Part model, mm, in its own coordinate system. A direction names the side the tool comes from. Round coordinates to 2 decimals unless told otherwise and drop trailing zeros. Write each loop counter-clockwise with the first axis right and the second up, starting at its lowest first coordinate (ties: lowest second). Pieces come first, ordered by that corner, then holes.
from build123d import *

# Parameters (mm, degrees)
BASE_BODY_DEPTH              = 37.5
UPPER_FLANGE_DEPTH           = 75
FLANGE_CORNER_FILLET_R13_A_R = 13
FLANGE_CORNER_FILLET_R13_B_R = 13
MOUNTING_HOLES_SKETCH_R      = 5
MOUNTING_HOLES_2X_10_DEPTH   = 75
SLOT_6MM_DEPTH               = 75
HANGER_PLATE_DEPTH           = 75
TAPER_CUT_DEPTH              = 75
EYE_BOSS_SKETCH_R            = 25
EYE_BOSS_DEPTH               = 10
EYE_HOLE_SKETCH_R            = 11.5
EYE_HOLE_23_DEPTH            = 10


with BuildPart() as part:
    # Base Profile Sketch → Base Body (new, symmetric)
    with BuildSketch(Plane.XY):
        Polygon((0, 11), (0, 21), (-27, 21), (-27, -21), (0, -21), (0, -11), (-17, -11), (-17, 11), align=None)
    extrude(amount=BASE_BODY_DEPTH, both=True)

    # Upper Flange Sketch → Upper Flange (add)
    with BuildSketch(Plane.XY.offset(37.5)):
        Polygon((0, 21), (0, 54), (10, 54), (10, 21), (10, 6.5), (0, 6.5), align=None)
    extrude(amount=-UPPER_FLANGE_DEPTH)

    # Flange Corner Fillet R13 A
    flange_corner_fillet_r13_a_edges = [part.edges().sort_by_distance(p)[0] for p in [
        (5, 54, 37.5),
    ]]
    fillet(flange_corner_fillet_r13_a_edges, radius=FLANGE_CORNER_FILLET_R13_A_R)

    # Flange Corner Fillet R13 B
    flange_corner_fillet_r13_b_edges = [part.edges().sort_by_distance(p)[0] for p in [
        (5, 54, -37.5),
    ]]
    fillet(flange_corner_fillet_r13_b_edges, radius=FLANGE_CORNER_FILLET_R13_B_R)

    # Mounting Holes Sketch → Mounting Holes 2xØ10 (cut)
    with BuildSketch(Plane.ZY):
        with Locations((24.5, 41)):
            Circle(MOUNTING_HOLES_SKETCH_R)
        with Locations((-24.5, 41)):
            Circle(MOUNTING_HOLES_SKETCH_R)
    extrude(amount=-MOUNTING_HOLES_2X_10_DEPTH, mode=Mode.SUBTRACT)

    # Slot Sketch → Slot 6mm (cut)
    with BuildSketch(Plane.ZY.offset(27)):
        with BuildLine():
            Line((-17.5, 6), (17.5, 6))
            ThreePointArc((17.5, 6), (23.5, 0), (17.5, -6))
            Line((17.5, -6), (-17.5, -6))
            ThreePointArc((-17.5, -6), (-23.5, 0), (-17.5, 6))
        make_face()
    extrude(amount=-SLOT_6MM_DEPTH, mode=Mode.SUBTRACT)

    # Hanger Plate Sketch → Hanger Plate (add)
    with BuildSketch(Plane.XY.offset(37.5)):
        Polygon((0, -6.5), (0, -21), (0, -73), (10, -73), (10, -21), (10, -6.5), align=None)
    extrude(amount=-HANGER_PLATE_DEPTH)

    # Taper Cut Sketch → Taper Cut (cut)
    with BuildSketch(Plane.ZY):
        Polygon((37.5, -73), (37.5, -21), (25, -73), align=None)
        Polygon((-25, -73), (-37.5, -21), (-37.5, -73), align=None)
    extrude(amount=-TAPER_CUT_DEPTH, mode=Mode.SUBTRACT)

    # Eye Boss Sketch → Eye Boss (add)
    with BuildSketch(Plane.ZY):
        with Locations((0, -73)):
            Circle(EYE_BOSS_SKETCH_R)
    extrude(amount=-EYE_BOSS_DEPTH)

    # Eye Hole Sketch → Eye Hole Ø23 (cut)
    with BuildSketch(Plane.ZY):
        with Locations(Location((0, -73, 0), (0, 0, 270))):
            Circle(EYE_HOLE_SKETCH_R)
    extrude(amount=-EYE_HOLE_23_DEPTH, mode=Mode.SUBTRACT)


solid = part.part
Q1. Drop flat-ended pins along their axis: P1, Ø18.5, axis at x = -10.5, z = 0, coming from the +Y side; P2, Ø3, axis at x = -23.5, z = 3.5, coming from the -Y side; P3, Ø8, axis at y = 41, z = -24.5, coming from the +X side; P4, Ø3, axis at y = -64.5, z = 7, coming from the +X side. Give the stop position or say it passes through.
Q2. Saw through at A-A, the plane x = -15. Write the cut outline in (y, z), and give its area (3 significant figures).
Q3. Two-plate mould, pull along X, no slides. Class faces 1 (the flat face through (5, -6.5, 1)), 2 (the flat face through (0, -50, 1)), 3 (the flat face through (0, -9, 1)), 4 (the flat face through (-17, -7, 1)): released by +X, released by -X, zero draft, split by the parting line, or undercut.
Q4. Saw through at D-D, the plane z = 0. Write the cut outline in (x, y), and give its area (3 significant figures).
Q5. Tool access for faces 5 (the flat face through (10, -43, 1)), 6 (the flat face through (-14, -21, 1)), 7 (the flat face through (0, 38, 1)), 8 (the flat face through (0, 9, 1)): list every direction of +Z, -Z, +X, -X, +Y, -Y with a clear straight run to the whole face (end or side of a thin tool).
Q6. Saw through at B-B, the plane z = -15.5. Write the cut outline in (x, y).
Q7. Wall check: line 1 (Y direction, x = -20.5, z = 13.5); line 2 (Y direction, x = -8, z = -32.5); line 3 (Z direction, x = 6.5, y = -73). Give the ranges that are in metal, low to high.
Q8. Saw through at C-C, the plane y = -68.5. Write the cut outline in (x, z).
Computed:
1. P1: stops at y = 21
1. P2: stops at y = -21
1. P3: passes through
1. P4: stops at x = 10
2. outline: (-21, -37.5) - (-11, -37.5) - (-11, 37.5) - (-21, 37.5) - close; (11, -37.5) - (21, -37.5) - (21, 37.5) - (11, 37.5) - close
2. area: 1,500 mm2
3. face 1: zero draft
3. face 2: released by -X
3. face 3: undercut
3. face 4: undercut
4. outline: (-27, -21) - (0, -21) - (0, -61.5) - (10, -61.5) - (10, -6.5) - (0, -6.5) - (0, -11) - (-17, -11) - (-17, -6) - (-27, -6) - close; (-27, 6) - (-17, 6) - (-17, 11) - (0, 11) - (0, 6.5) - (10, 6.5) - (10, 54) - (0, 54) - (0, 21) - (-27, 21) - close; (0, -98) - (10, -98) - (10, -84.5) - (0, -84.5) - close
4. area: 1,800 mm2
5. face 5: +Z, -Z, +X, +Y, -Y
5. face 6: +Z, -Z, -X, -Y
5. face 7: +Z, -Z, -X, +Y
5. face 8: +Z, -Z
6. outline: (-27, -21) - (0, -21) - (0, -92.62) - (10, -92.62) - (10, -6.5) - (0, -6.5) - (0, -11) - (-17, -11) - (-17, -6) - (-27, -6) - close; (-27, 6) - (-17, 6) - (-17, 11) - (0, 11) - (0, 6.5) - (10, 6.5) - (10, 54) - (0, 54) - (0, 21) - (-27, 21) - close
7. line 1: y = -21 to -6, 6 to 21
7. line 2: y = -21 to -11, 11 to 21
7. line 3: z = -25 to -11.5, 11.5 to 25
8. outline: (0, -26.08) - (10, -26.08) - (10, -10.58) - (0, -10.58) - close; (0, 10.58) - (10, 10.58) - (10, 26.08) - (0, 26.08) - close
